Build history of the part. All positions in model axes, mm. Coordinates: 2 decimals unless noted, no trailing zeros. Order: outer loops, then holes, each group sorted by start corner. A loop starts at its lowest first (then second) coordinate and runs counter-clockwise, first axis right, second up. Notation, with made-up numbers: (12.5, -39) - (45.5, -39) arc R9 cw to (45.5, -24) - close; hole circle Ø11 at (36, 13.5). An arc over 180 degrees is marked (long way). Write each question's results on one line, items separated by ' | '.
from build123d import *

# Parameters (mm, degrees)
SKETCH1_W                     = 560
SKETCH1_H                     = 670
BOSS_EXTRUDE1_DEPTH           = 12
SKETCH3_R                     = 4.25
SKETCH3_R_2                   = 0.639613625
CUT_EXTRUDE1_DEPTH            = 12
MIRROR2_COPY_1_SKETCH_R       = 4.25
MIRROR2_COPY_1_SKETCH_R_2     = 0.639613625
MIRROR2_COPY_1_DEPTH          = 12
CSK_FOR_M6_SFHCS1_D           = 6.6
CSK_FOR_M6_SFHCS1_CSINK_D     = 13.44
CSK_FOR_M6_SFHCS1_CSINK_ANGLE = 90
SKETCH10_W                    = 65.8
SKETCH10_H                    = 611
CUT_EXTRUDE2_DEPTH            = 111
SKETCH11_W                    = 31.663111861
SKETCH11_H                    = 60.455114524
CUT_EXTRUDE3_DEPTH            = 55


with BuildPart() as part:
    # Sketch1 → Boss-Extrude1 (new body)
    with BuildSketch(Plane(origin=(0, 0, 0), x_dir=(1, 0, 0), z_dir=(0, 1, 0))):
        Rectangle(SKETCH1_W, SKETCH1_H)
    extrude(amount=BOSS_EXTRUDE1_DEPTH)

    # Sketch3 → Cut-Extrude1 (cut)
    with BuildSketch(Plane(origin=(0, 12, 0), x_dir=(1, 0, 0), z_dir=(0, 1, 0))):
        with Locations(Location((210, 240, 0), (0, 0, 270))):
            Circle(SKETCH3_R)
        with Locations(Location((70, 240, 0), (0, 0, 270))):
            Circle(SKETCH3_R)
        with Locations(Location((210, 120, 0), (0, 0, 270))):
            Circle(SKETCH3_R)
        with Locations(Location((70, 120, 0), (0, 0, 270))):
            Circle(SKETCH3_R)
        with Locations(Location((70, 0, 0), (0, 0, 270))):
            Circle(SKETCH3_R)
        with Locations(Location((210, 0, 0), (0, 0, 270))):
            Circle(SKETCH3_R)
        with Locations(Location((0, 0, 0), (0, 0, 270))):
            Circle(SKETCH3_R_2)
    cut_extrude1 = extrude(amount=-CUT_EXTRUDE1_DEPTH, mode=Mode.SUBTRACT)

    # Mirror1: Cut-Extrude1 across plane
    add(cut_extrude1.mirror(Plane(origin=(0, 0, 0), x_dir=(0, 0, 1), z_dir=(1, 0, 0))), mode=Mode.SUBTRACT)

    # Mirror2: Cut-Extrude1 across plane
    add(cut_extrude1.mirror(Plane.XY), mode=Mode.SUBTRACT)

    # Mirror2 copy 1 sketch → Mirror2 copy 1 (cut)
    with BuildSketch(Plane(origin=(0, 12, 0), x_dir=(-1, 0, 0), z_dir=(0, 1, 0))):
        with Locations(Location((210, 240, 0), (0, 0, 270))):
            Circle(MIRROR2_COPY_1_SKETCH_R)
        with Locations(Location((70, 240, 0), (0, 0, 270))):
            Circle(MIRROR2_COPY_1_SKETCH_R)
        with Locations(Location((210, 120, 0), (0, 0, 270))):
            Circle(MIRROR2_COPY_1_SKETCH_R)
        with Locations(Location((70, 120, 0), (0, 0, 270))):
            Circle(MIRROR2_COPY_1_SKETCH_R)
        with Locations(Location((70, 0, 0), (0, 0, 270))):
            Circle(MIRROR2_COPY_1_SKETCH_R)
        with Locations(Location((210, 0, 0), (0, 0, 270))):
            Circle(MIRROR2_COPY_1_SKETCH_R)
        with Locations(Location((0, 0, 0), (0, 0, 270))):
            Circle(MIRROR2_COPY_1_SKETCH_R_2)
    extrude(amount=-MIRROR2_COPY_1_DEPTH, mode=Mode.SUBTRACT)

    # CSK for M6 SFHCS1 (through all)
    with Locations(Plane(origin=(0, 12, 0), x_dir=(1, 0, 0), z_dir=(0, 1, 0))):
        with Locations((0, 0), (260, 0), (0, 325), (260, 325), (0, -325), (-260, 0), (-260, 325), (-260, -325), (260, -325)):
            CounterSinkHole(CSK_FOR_M6_SFHCS1_D / 2, CSK_FOR_M6_SFHCS1_CSINK_D / 2, counter_sink_angle=CSK_FOR_M6_SFHCS1_CSINK_ANGLE)

    # Sketch10 → Cut-Extrude2 (cut)
    with BuildSketch(Plane(origin=(0, 12, 0), x_dir=(1, 0, 0), z_dir=(0, 1, 0))):
        with Locations((1.4, -10)):
            Rectangle(SKETCH10_W, SKETCH10_H)
    extrude(amount=-CUT_EXTRUDE2_DEPTH, mode=Mode.SUBTRACT)

    # Sketch11 → Cut-Extrude3 (cut)
    with BuildSketch(Plane(origin=(0, 12, 0), x_dir=(1, 0, 0), z_dir=(0, 1, 0))):
        with Locations((-46.831555931, -186)):
            Rectangle(SKETCH11_W, SKETCH11_H)
    cut_extrude3 = extrude(amount=-CUT_EXTRUDE3_DEPTH, mode=Mode.SUBTRACT)

    # Mirror3: Cut-Extrude3 across plane
    add(cut_extrude3.mirror(Plane.XY), mode=Mode.SUBTRACT)


solid = part.part
1. Probe line 1 (X direction, y = 6.25, z = -240); line 2 (Z direction, x = -70, y = 2.5); line 3 (X direction, y = 2.5, z = -208.5). List the from-to ranges inside material, lowest first.
Solved:
line 1: x = -280 to -214.25, -205.75 to -74.25, -65.75 to -31.5, 34.3 to 65.75, 74.25 to 205.75, 214.25 to 280 | line 2: z = -335 to -244.25, -235.75 to -124.25, -115.75 to -4.25, 4.25 to 115.75, 124.25 to 235.75, 244.25 to 335 | line 3: x = -280 to -62.66, 34.3 to 280
2. Band-saw the part on A-A on z = -187. Give the cut face in (x, y).
Solved:
outline: (-280, 0) - (-62.66, 0) - (-62.66, 12) - (-280, 12) - close; (34.3, 0) - (280, 0) - (280, 12) - (34.3, 12) - close
3. Two-plate mould, pull along Z, no slides. Class faces 1 (the face through (-1.863, 8.746, -327.923)), 2 (the face through (58, 12, -5)): +Z half, -Z half, draft (parallel to the pull), parting line (faces both ways), or undercut.
Solved:
face 1: undercut | face 2: draft
4. Drop flat-ended pins along their axis: pin 1 Ø7.5 at (x, z) = (0, 325) entering from +Y; pin 2 Ø7 at (x, z) = (-70, 240) entering from -Y; pin 3 Ø10 at (x, z) = (-70, 0) entering from -Y. Give the stop position or say it passes through.
Solved:
pin 1: stops at y = 9.03 | pin 2: passes through | pin 3: stops at y = 0
5. Band-saw the part on B-B on y = 5. Give the number of separate pieces and of enclosed holes in the cut face, then the cut area to 3 significant figures.
Solved:
separate pieces: 1 | enclosed holes: 29 | area: 330,000 mm2
6. Band-saw the part on C-C on z = -20. Give the cut face in (x, y), then the cut area to 3 significant figures.
Solved:
outline: (-280, 0) - (-31.5, 0) - (-31.5, 12) - (-280, 12) - close; (34.3, 0) - (280, 0) - (280, 12) - (34.3, 12) - close | area: 5,930 mm2
